Could you check a few things on this drawing? It's one solid part, dimensions in mm from its lowest x, y, z. Coordinates: 2 decimals unless noted, no trailing zeros. Order: outer loops, then holes, each group sorted by start corner. A loop starts at its lowest first (then second) coordinate and runs counter-clockwise, first axis right, second up. Notation, with made-up numbers: (69, -1.5) -> (112, -1.5) arc R21 cw to (112, 17.5) -> close; hole circle Ø8 at (84.25, 85.25). An arc over 180 degrees is marked (long way). Use a Markdown table: item, result. Add a question column.
1. Suppose I cut it at A-A, the plane z = 4. List the corners of the cut face in (x, y) for me, then the cut area to 3 significant figures.
2. For pin 1 Ø4.5 at (x, z) = (86, 4) entering from -Y; pin 2 Ø2.5 at (x, z) = (4, 4) entering from -Y; pin 3 Ø3.5 at (x, z) = (4, 66) entering from +Y, each with a flat end and sliding along its axis, tell me the tip position at first contact or that it passes through.
3. If I drill on line 1 along Z through (x, y) = (4, 1.2); line 2 along X through (y, z) = (3.95, 4); line 3 along X through (y, z) = (0.75, 66), over which ranges is the centre line in solid material (lowest first)? Write a range as from..to.
4. Suppose I cut it at B-B, the plane x = 86. List the corners of the cut face in (y, z) for me.
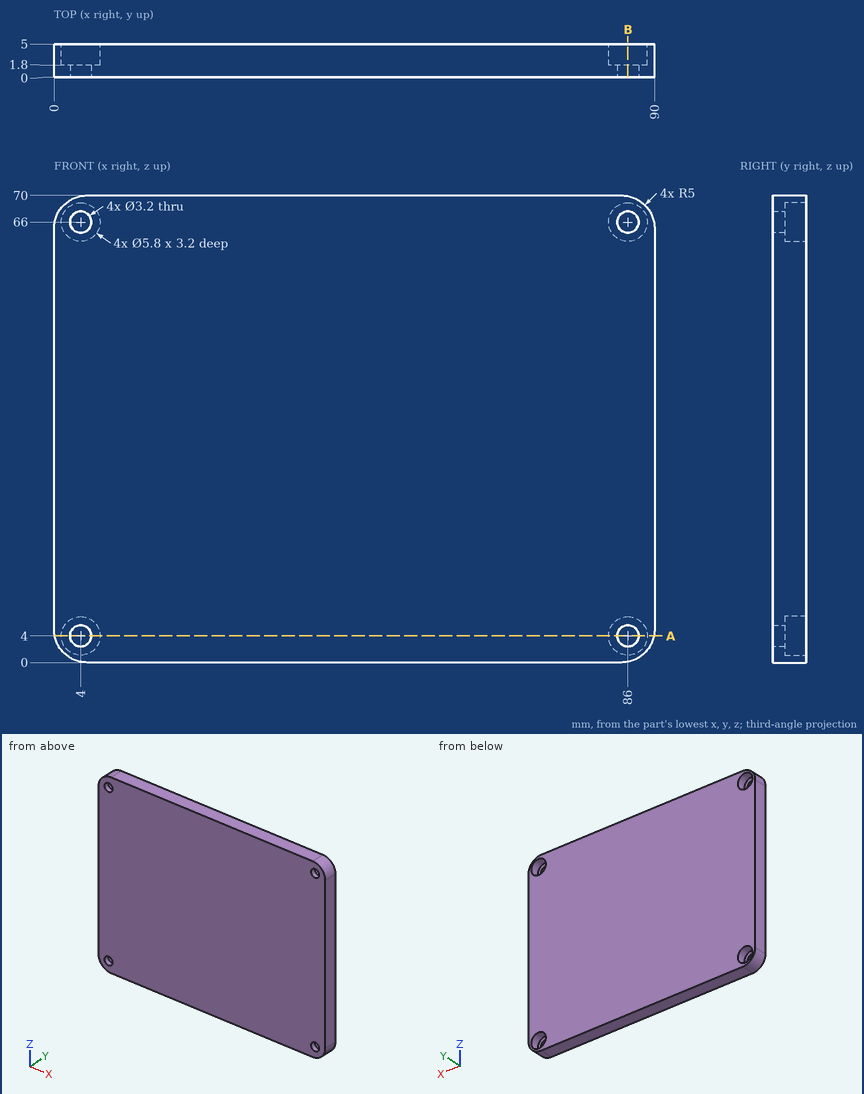
Worked out:
| question | item | result |
|---|---|---|
| 1 | outline | (0.1, 0) -> (2.4, 0) -> (2.4, 1.8) -> (1.1, 1.8) -> (1.1, 5) -> (0.1, 5) -> close; (5.6, 0) -> (84.4, 0) -> (84.4, 1.8) -> (83.1, 1.8) -> (83.1, 5) -> (6.9, 5) -> (6.9, 1.8) -> (5.6, 1.8) -> close; (87.6, 0) -> (89.9, 0) -> (89.9, 5) -> (88.9, 5) -> (88.9, 1.8) -> (87.6, 1.8) -> close |
| 1 | area | 400 mm² |
| 2 | pin 1 | stops at y = 0 |
| 2 | pin 2 | passes through |
| 2 | pin 3 | stops at y = 1.8 |
| 3 | line 1 | z = 0.1..2.4, 5.6..64.4, 67.6..69.9 |
| 3 | line 2 | x = 0.1..1.1, 6.9..83.1, 88.9..89.9 |
| 3 | line 3 | x = 0.1..2.4, 5.6..84.4, 87.6..89.9 |
| 4 | outline | (0, 0.1) -> (5, 0.1) -> (5, 1.1) -> (1.8, 1.1) -> (1.8, 2.4) -> (0, 2.4) -> close; (0, 5.6) -> (1.8, 5.6) -> (1.8, 6.9) -> (5, 6.9) -> (5, 63.1) -> (1.8, 63.1) -> (1.8, 64.4) -> (0, 64.4) -> close; (0, 67.6) -> (1.8, 67.6) -> (1.8, 68.9) -> (5, 68.9) -> (5, 69.9) -> (0, 69.9) -> close |
